from build123d import *

# Parameters (mm, degrees)
CUT_EXTRUDE1_DEPTH = 5
CIRPATTERN1_COUNT  = 4


with BuildPart() as part:
    # Sketch1 → Revolve1 (revolve)
    with BuildSketch(Plane.XY):
        Polygon((-3.366724667, 20.25), (0, 29.5), (0, 32), (-19, 32), (-19, 30.5), (-23, 30.5), (-23, 32), (-23, 37), (-35, 37), (-35, 28), (-29, 28), (-29, 22), (-28, 21), (-26, 21), (-26, 20.25), align=None)
    revolve(axis=Axis((0, 0, 0), (-1, 0, 0)))

    # Sketch2 → Cut-Extrude1 (cut)
    with BuildSketch(Plane.ZY.offset(35)):
        with BuildLine():
            ThreePointArc((3, 36.878177829), (0, 37), (-3, 36.878177829))
            Line((-3, 36.878177829), (-3, 27.838821814))
            ThreePointArc((-3, 27.838821814), (0, 28), (3, 27.838821814))
            Line((3, 27.838821814), (3, 36.878177829))
        make_face()
    cut_extrude1 = extrude(amount=-CUT_EXTRUDE1_DEPTH, mode=Mode.SUBTRACT)

    # CirPattern1: Cut-Extrude1 ×4 about axis
    cirpattern1_axis = Axis((0, 0, 0), (1, 0, 0))
    for i in range(1, CIRPATTERN1_COUNT):
        add(cut_extrude1.rotate(cirpattern1_axis, i * 360 / CIRPATTERN1_COUNT), mode=Mode.SUBTRACT)


solid = part.part
CAD build for the part. Positions are in the model's coordinates, mm. A direction names the side the tool comes from. Coordinates: 2 decimals unless noted, no trailing zeros. Write each loop counter-clockwise with the first axis right and the second up, starting at its lowest first coordinate (ties: lowest second). Pieces come first, ordered by that corner, then holes. Notation, with made-up numbers: M 32,88 L 76,88 A9 cw 76,97 Z; hole C 52,44 d2. An arc over 180 degrees is marked long. Answer as a JSON object with one key per item and string values. Group by question number.
1) Mould opens along X. For faces 1 (the face through (-33, 32, -3)), 2 (the face through (-19, 25.9, 16.4)), 3 (the face through (-3.156, -4.515, 20.333)), 4 (the face through (-30, -32, 0)) say: +X half, -X half, draft (parallel to the pull), parting line (faces both ways), or undercut.
2) Saw through at D-D (x = -7). Write the cut outline in (y, z).
3) Tool access for faces 5 (the face through (-30, 32, 0)), 6 (the face through (-33, 3, -32)), 7 (the face through (-31.958, 26.707, -8.41)): list every direction of +Z, -Z, +X, -X, +Y, -Y with a clear straight run to the whole face (end or side of a thin tool).
4) Saw through at B-B (x = -32). Write the cut outline in (y, z), plus the area to 3 significant figures.
5) Saw through at A-A (y = 0). Write the cut outline in (x, z), plus the area to 3 significant figures.
6) Wall check: line 1 (X direction, y = -15, z = 27); line 2 (Z direction, x = -27, y = 0). Give the ranges that are in metal, low to high. Write a range as from..to.
7) Pin check, flat tips, straight feed: pin 1 Ø4 at (x, z) = (-32.5, 34.5) entering from +Y; pin 2 Ø10 at (y, z) = (21, 5) entering from +X; pin 3 Ø1.8 at (y, z) = (30.5, 1) entering from -X. Stop position of each tip, or through.
Values follow:
{
 "1": {"face 1": "draft", "face 2": "undercut", "face 3": "+X half", "face 4": "-X half"},
 "2": {"outline": "C 0,0 d64; hole C 0,0 d40.5"},
 "3": {"face 5": "-X, +Y, -Y", "face 6": "+Z, -Z, -X", "face 7": "-X"},
 "4": {"outline": "M -36.88,-3 A37 ccw -3,-36.88 L -3,-27.84 A28 cw -27.84,-3 Z; M -36.88,3 L -27.84,3 A28 cw -3,27.84 L -3,36.88 A37 ccw Z; M 3,-36.88 A37 ccw 36.88,-3 L 27.84,-3 A28 cw 3,-27.84 Z; M 3,27.84 A28 cw 27.84,3 L 36.88,3 A37 ccw 3,36.88 Z", "area": "1,620 mm2"},
 "5": {"outline": "M -30,-37 L -23,-37 L -23,-30.5 L -19,-30.5 L -19,-32 L 0,-32 L 0,-29.5 L -3.37,-20.25 L -26,-20.25 L -26,-21 L -28,-21 L -29,-22 L -29,-28 L -30,-28 Z; M -30,28 L -29,28 L -29,22 L -28,21 L -26,21 L -26,20.25 L -3.37,20.25 L 0,29.5 L 0,32 L -19,32 L -19,30.5 L -23,30.5 L -23,37 L -30,37 Z", "area": "711 mm2"},
 "6": {"line 1": "x = -35..-23, -19..0", "line 2": "z = -37..-21, 21..37"},
 "7": {"pin 1": "stops at y = 17.68", "pin 2": "stops at x = -1.06", "pin 3": "stops at x = -30"}
}
